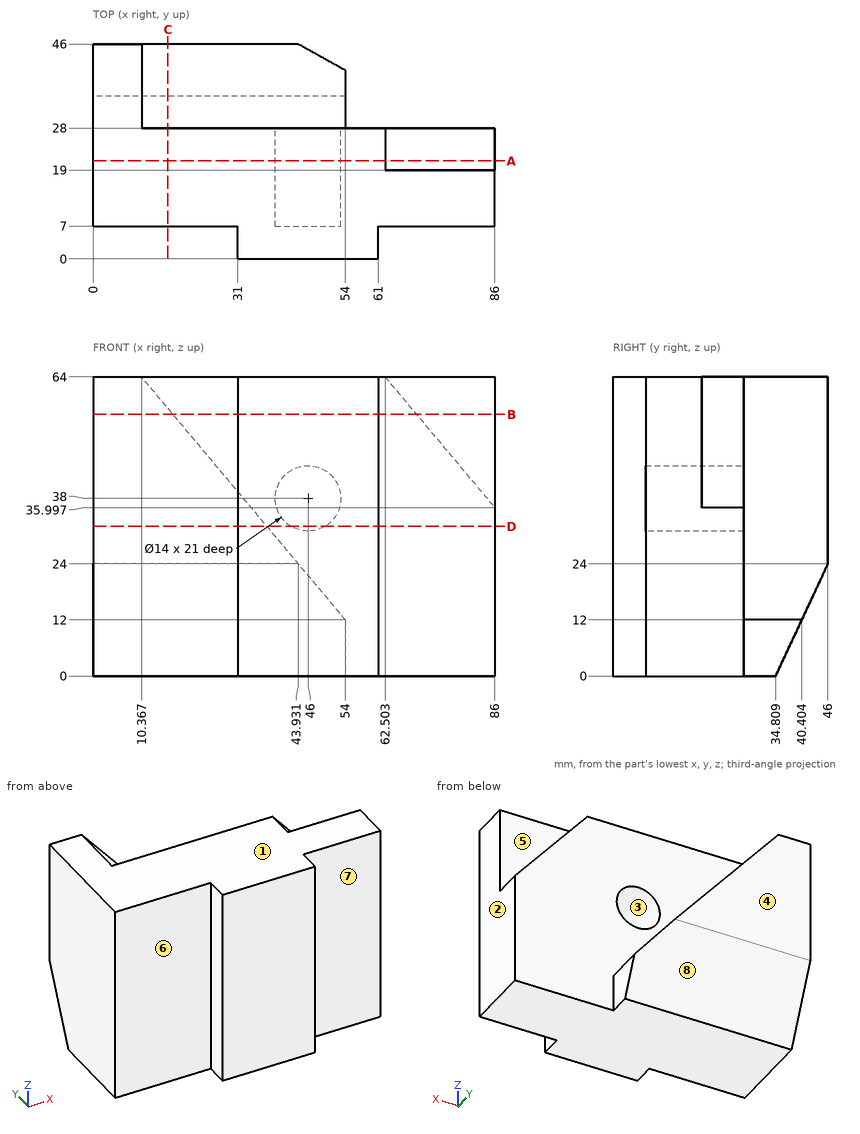
The figure shows three views and two pictorial views of one solid part (mm, origin at its lowest corner). Answer the questions. A direction names the side the tool comes from. Coordinates: 2 decimals unless noted, no trailing zeros. Loops run counter-clockwise (first coordinate to the right, second up) from the corner with the lowest first, then second, coordinate; pieces in that order, holes last. Notation, with made-up numbers: (82.25, -15.75) -> (119.25, -15.75) arc R13 cw to (119.25, -4.75) -> close; hole circle Ø10 at (56.25, -13). An arc over 180 degrees is marked (long way). Use one line per item in the form item = value. Start each with the question number.
Item 1: A tool of negligible diameter and unlimited length cuts with its end or side. For the marked faces 4, 5, 6, 7 and 8, from which of +Z, -Z, +X, -X, +Y, -Y can it reach the whole face along a straight path? Write none if from no direction.
Item 2: The part is cut by section B-B on z = 56. Determine the outline of the cut face in (x, y) (1 decimal).
Item 3: The part is cut by section D-D on z = 32. Determine the outline of the cut face in (x, y) (1 decimal), then the cut area to 3 significant figures.
Item 4: The part is cut by section C-C on x = 16. Determine the outline of the cut face in (y, z).
Item 5: The part is cut by section A-A on y = 21. Determine the outline of the cut face in (x, z).
Item 6: Flat-ended cylindrical pins translate along their axes: pin 1 Ø6 at (y, z) = (36.5, 5) entering from +X; pin 2 Ø8 at (x, z) = (40, 43.5) entering from +Y; pin 3 Ø1 at (x, z) = (30, 37) entering from -Y; pin 4 Ø1 at (x, y) = (11.5, 5.5) entering from +Z. Find the tip coordinate at first contact, or state that the pin passes through.
Item 7: The mould has two halves that part along X. Classify the marked faces 1, 2 and 3: released by +X, released by -X, zero draft, split by the parting line, or undercut.
Item 8: Consider L1, parallel to X at y = 16.75, z = 38; L2, parallel to Z at x = 46, y = 16; L3, parallel to Y at x = 41.5, z = 40.5. Determine where each line is inside the solid, lowest interval first. Write a range as [from, to].
Answer key:
q1.face_4 = +Z, -Z, +X, -X, +Y
q1.face_5 = +Z, +X, +Y
q1.face_6 = +Z, -Z, -X, -Y
q1.face_7 = +Z, -Z, +X, -Y
q1.face_8 = -Z, +X, -X, +Y
q2.outline = (0, 7) -> (31, 7) -> (31, 0) -> (61, 0) -> (61, 7) -> (86, 7) -> (86, 19) -> (69.2, 19) -> (69.2, 28) -> (17.1, 28) -> (17.1, 46) -> (0, 46) -> close
q3.outline = (0, 7) -> (31, 7) -> (31, 0) -> (61, 0) -> (61, 7) -> (86, 7) -> (86, 28) -> (49.6, 28) -> (49.6, 7) -> (42.4, 7) -> (42.4, 28) -> (37.2, 28) -> (37.2, 46) -> (0, 46) -> close
q3.area = 2,530 mm2
q4.outline = (7, 0) -> (34.81, 0) -> (46, 24) -> (46, 57.29) -> (28, 57.29) -> (28, 64) -> (7, 64) -> close
q5.outline = (0, 0) -> (86, 0) -> (86, 36) -> (62.5, 64) -> (0, 64) -> close; hole circle Ø14 at (46, 38)
q6.pin_1 = 54
q6.pin_2 = 28
q6.pin_3 = 7
q6.pin_4 = through
q7.face_1 = zero draft
q7.face_2 = released by +X
q7.face_3 = undercut
q8.L1 = [0, 39], [53, 86]
q8.L2 = [0, 31], [45, 64]
q8.L3 = [0, 7]
